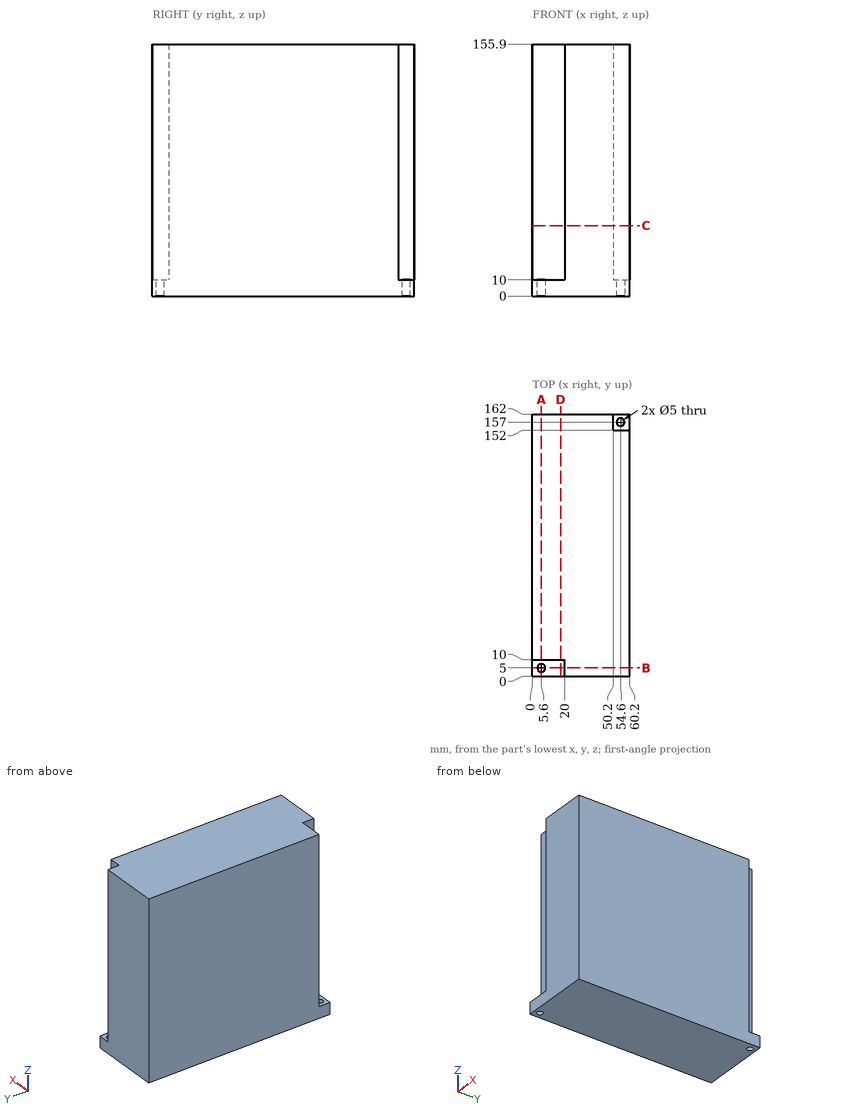
Print and shaded views of the part. All mm, measured from the part's lowest x, y and z. Give positions to 0.01 mm unless a question says otherwise; leave off trailing zeros. Order: outer loops, then holes, each group sorted by start corner. A loop starts at its lowest first (then second) coordinate and runs counter-clockwise, first axis right, second up. Notation, with made-up numbers: M 19.25,69 L 49.25,69 A21 cw 49.25,100 Z; hole C 36.5,70.25 d5. An arc over 180 degrees is marked long. Use one line per item in the form item = value.
Q1. Slice it at C-C, the plane z = 43.5. Write the cut outline in (x, y), and give its area (3 significant figures).
Conclusion:
outline = M 0,10 L 20,10 L 20,0 L 60.2,0 L 60.2,152 L 50.2,152 L 50.2,162 L 0,162 Z
area = 9,450 mm2
Q2. Slice it at D-D, the plane x = 17.5. Write the cut outline in (y, z).
Conclusion:
outline = M 0,0 L 162,0 L 162,155.9 L 10,155.9 L 10,10 L 0,10 Z
Q3. Wall check: probe 1 along Y at (x, z) = (54.6, 5.25); probe 2 along Y at (x, z) = (5.6, 2.75); probe 3 along X at (y, z) = (157, 3). Give the ranges that are in metal, low to high.
Conclusion:
probe_1 = 0 to 154.5, 159.5 to 162
probe_2 = 0 to 2.5, 7.5 to 162
probe_3 = 0 to 52.1, 57.1 to 60.2
Q4. Slice it at A-A, the plane x = 5.6. Write the cut outline in (y, z).
Conclusion:
outline = M 0,0 L 2.5,0 L 2.5,10 L 0,10 Z; M 7.5,0 L 162,0 L 162,155.9 L 10,155.9 L 10,10 L 7.5,10 Z
Q5. Slice it at B-B, the plane y = 5. Write the cut outline in (x, z), and give its area (3 significant figures).
Conclusion:
outline = M 0,0 L 3.1,0 L 3.1,10 L 0,10 Z; M 8.1,0 L 60.2,0 L 60.2,155.9 L 20,155.9 L 20,10 L 8.1,10 Z
area = 6,420 mm2
Q6. Pin check, flat tips, straight feed: P1, Ø5, axis at x = 8, y = 5.5, coming from the +Z side; P2, Ø5, axis at y = 4, z = 82.5, coming from the -X side; P3, Ø5, axis at y = 158, z = 53, coming from the +X side; P4, Ø3, axis at x = 5.6, y = 5, coming from the -Z side. Stop position of each tip, or through.
Conclusion:
P1 = 10
P2 = 20
P3 = 50.2
P4 = through
